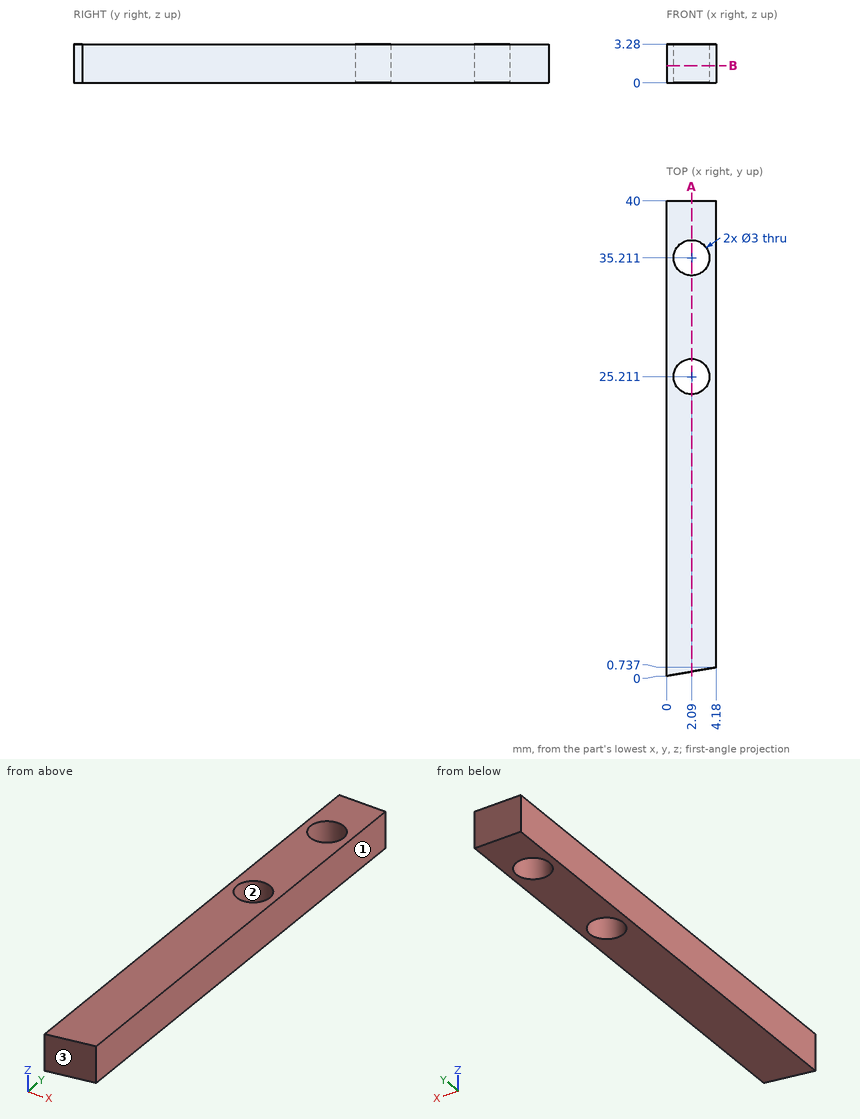
Verification items for this drawing (mm, ordinates from the low corner). Give positions to 0.01 mm unless a question says otherwise; leave off trailing zeros. Loops run counter-clockwise (first coordinate to the right, second up) from the corner with the lowest first, then second, coordinate; pieces in that order, holes last. Notation, with made-up numbers: M -35.75,27.5 L -18.75,27.5 A26 ccw -18.75,46.5 Z; hole C -26.75,40.25 d8. An arc over 180 degrees is marked long. Return JSON: item names as keys, results as strings. Group by question number.
1. Mould release check, pull along Y, two halves, no side actions. Record for the marked faces 1, 2 and 3: released by +Y, released by -Y, zero draft, split by the parting line, or undercut.
2. Go/stop test with a flat-tipped pin: pin 1 (1.8 mm diameter, centred on x = 2.09, y = 25.21, fed in from -Z). Record where the tip stops, or that it passes through.
3. Thickness scan on L1, parallel to Y at x = 0.95, z = 1.7 (1 decimal); L2, parallel to Y at x = 2.09, z = 1.15; L3, parallel to Y at x = 0.55, z = 2.95. Record the ranges inside material, lowest first.
4. Cross-section at A-A on x = 2.09. Record the boundary of the cut face in (y, z).
5. Cross-section at B-B on z = 1.45. Record the boundary of the cut face in (x, y).
Return value:
{
 "1": {"face 1": "zero draft", "face 2": "undercut", "face 3": "released by -Y"},
 "2": {"pin 1": "through"},
 "3": {"L1": "0.2 to 24.2, 26.2 to 34.2, 36.2 to 40", "L2": "0.37 to 23.71, 26.71 to 33.71, 36.71 to 40", "L3": "0.1 to 40"},
 "4": {"outline": "M 0.37,0 L 23.71,0 L 23.71,3.28 L 0.37,3.28 Z; M 26.71,0 L 33.71,0 L 33.71,3.28 L 26.71,3.28 Z; M 36.71,0 L 40,0 L 40,3.28 L 36.71,3.28 Z"},
 "5": {"outline": "M 0,0 L 4.18,0.74 L 4.18,40 L 0,40 Z; hole C 2.09,25.21 d3; hole C 2.09,35.21 d3"}
}
